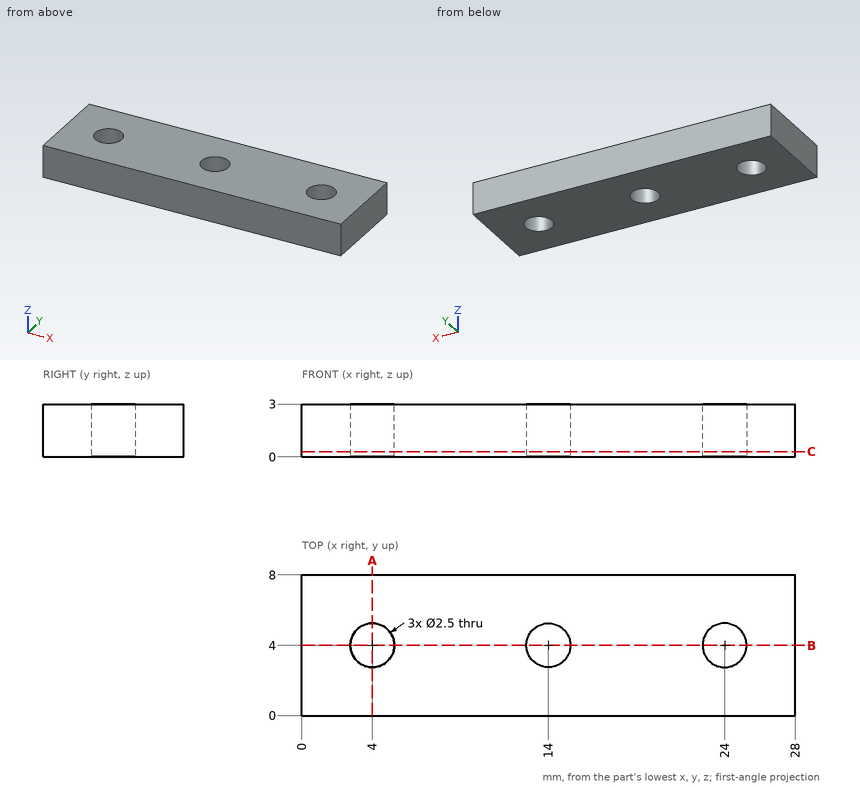
Input: dimensioned drawing with shaded views. Units: mm. Origin: part minimum x, y, z. Coordinates: 2 decimals unless noted, no trailing zeros. Write each loop counter-clockwise with the first axis right and the second up, starting at its lowest first coordinate (ties: lowest second). Pieces come first, ordered by that corner, then holes. Notation, with made-up numbers: M 5,33.5 L 64,33.5 A25 cw 64,55.5 Z; hole C 40,-24.75 d4. An arc over 180 degrees is marked long. Answer as a JSON object with one key per item and string values. Group by question number.
(1) Contact query for a flat-ended pin moving along its axis: P1, Ø1.5, axis at y = 1.5, z = 2.5, coming from the -X side. Output: stop coordinate, or through.
(2) Section A-A on x = 4. Output: boundary loops of the cut face in (y, z), plus the area to 3 significant figures.
(3) Ray query, line 1 along X through (y, z) = (3, 2.3); line 2 along Y through (x, z) = (24, 2.35); line 3 along X through (y, z) = (4.75, 0.7). Return the intervals inside material, ascending. Write a range as [from, to].
(4) Section C-C on z = 0.3. Output: boundary loops of the cut face in (x, y), plus the area to 3 significant figures.
(5) Section B-B on y = 4. Output: boundary loops of the cut face in (x, z), plus the area to 3 significant figures.
Result set:
{
 "1": {"P1": "stops at x = 0"},
 "2": {"outline": "M 0,0 L 2.75,0 L 2.75,3 L 0,3 Z; M 5.25,0 L 8,0 L 8,3 L 5.25,3 Z", "area": "16.5 mm2"},
 "3": {"line 1": "x = [0, 3.25], [4.75, 13.25], [14.75, 23.25], [24.75, 28]", "line 2": "y = [0, 2.75], [5.25, 8]", "line 3": "x = [0, 3], [5, 13], [15, 23], [25, 28]"},
 "4": {"outline": "M 0,0 L 28,0 L 28,8 L 0,8 Z; hole C 4,4 d2.5; hole C 14,4 d2.5; hole C 24,4 d2.5", "area": "209 mm2"},
 "5": {"outline": "M 0,0 L 2.75,0 L 2.75,3 L 0,3 Z; M 5.25,0 L 12.75,0 L 12.75,3 L 5.25,3 Z; M 15.25,0 L 22.75,0 L 22.75,3 L 15.25,3 Z; M 25.25,0 L 28,0 L 28,3 L 25.25,3 Z", "area": "61.5 mm2"}
}
